Study the drawing (mm; zero at the part's minimum x, y, z) and answer. A direction names the side the tool comes from. Give positions to 0.01 mm unless a question says otherwise; leave off trailing zeros. Order: outer loops, then holes, each group sorted by start corner. A loop starts at its lowest first (then second) coordinate and runs counter-clockwise, first axis right, second up. Notation, with made-up numbers: (71, 56.25) -> (121, 56.25) arc R29 ccw to (121, 91.25) -> close; hole circle Ø3 at (-4, 28.25). An arc over 180 degrees is marked (long way). Use a Markdown table: item, result. Add a question column.
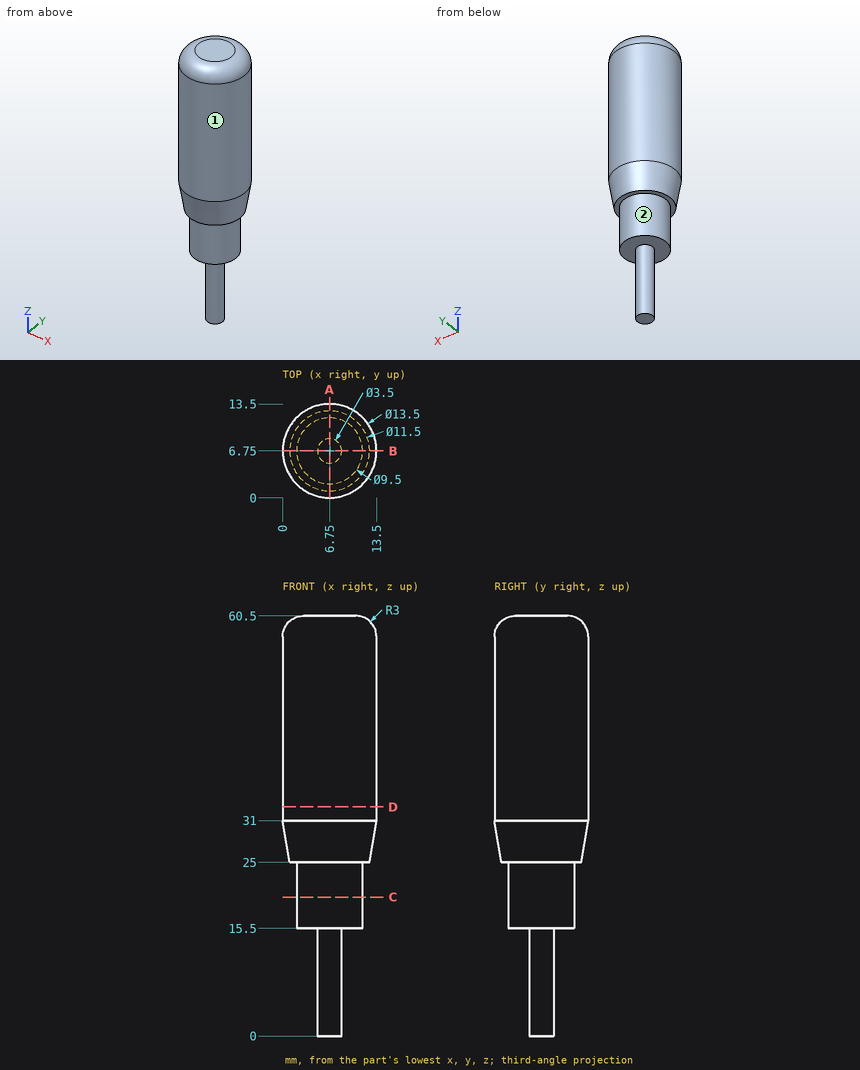
1) Which of the six approach directions +Z, -Z, +X, -X, +Y, -Y give full straight-line access (tool end or side, diameter ignored) to the marked faces 1 and 2?
2) The part is cut by section C-C, the plane z = 20. Determine the outline of the cut face in (x, y), then the cut area to 3 significant figures.
3) The part is cut by section D-D, the plane z = 33. Determine the outline of the cut face in (x, y), then the cut area to 3 significant figures.
4) Straight lines are drawn through the part: line 1 (Z direction, x = 7.5, y = 3); line 2 (Y direction, x = 7, z = 51); line 3 (Y direction, x = 2.25, z = 51). For each, find the intervals that lie inside material, in ascending order.
5) The part is cut by section A-A, the plane x = 6.75. Determine the outline of the cut face in (y, z), then the cut area to 3 significant figures.
6) Flat-ended cylindrical pins translate along their axes: pin 1 (1.5 mm diameter, centred on x = 1.5, y = 6, fed in from +Z); pin 2 (5 mm diameter, centred on x = 3, y = 10, fed in from -Z); pin 3 (3 mm diameter, centred on x = 5.5, z = 17, fed in from +Y). Find the tip coordinate at first contact, or state that the pin passes through.
A:
| question | item | result |
|---|---|---|
| 1 | face 1 | +Z, -Z |
| 1 | face 2 | -Z |
| 2 | outline | circle Ø9.5 at (6.75, 6.75) |
| 2 | area | 70.9 mm^2 |
| 3 | outline | circle Ø13.5 at (6.75, 6.75) |
| 3 | area | 143 mm^2 |
| 4 | line 1 | 15.5 to 60.5 |
| 4 | line 2 | 0 to 13.5 |
| 4 | line 3 | 1.72 to 11.78 |
| 5 | outline | (0, 31) -> (1, 25) -> (2, 25) -> (2, 15.5) -> (5, 15.5) -> (5, 0) -> (8.5, 0) -> (8.5, 15.5) -> (11.5, 15.5) -> (11.5, 25) -> (12.5, 25) -> (13.5, 31) -> (13.5, 57.5) arc R3 ccw to (10.5, 60.5) -> (3, 60.5) arc R3 ccw to (0, 57.5) -> close |
| 5 | area | 614 mm^2 |
| 6 | pin 1 | z = 60.39 |
| 6 | pin 2 | z = 15.5 |
| 6 | pin 3 | y = 11.5 |
